Could you check a few things on this model? Use its own coordinates, in mm. Give positions to 0.01 mm unless a question says otherwise; leave off trailing zeros. Loops run counter-clockwise (first coordinate to the right, second up) from the corner with the lowest first, then second, coordinate; pieces in that order, holes last. Notation, with made-up numbers: (26, 41) - (43, 41) arc R23 ccw to (43, 69) - close; hole circle Ø1 at (52, 8.5). An arc over 180 degrees is marked (long way). One line per item, written item: value. Start each with the question number.
Q1. If I drill on line 1 (X direction, y = 59.7, z = 0.75); line 2 (Y direction, x = 0, z = 0.2); line 3 (X direction, y = 58.6, z = 0.2), over which ranges is the centre line in solid material (lowest first)? Write a range as from..to.
Q2. I'm going to push a flat-ended pin straight in: P1, Ø2, axis at x = 0, y = 59.56, coming from the +Z side. Where does the tip first touch, or does it pass through?
Q3. I want a section at A-A (x = 0). Please give me the cut outline in (y, z).
Q4. I want a section at B-B (z = 0.4). Please give me the cut outline in (x, y), then the cut area to 3 significant figures.
```python
from build123d import *

# Parameters (mm, degrees)
SKETCH1_W           = 119.309628318
SKETCH1_H           = 4.994236566
BOSS_EXTRUDE1_DEPTH = 1
SKETCH2_R           = 1.25
CUT_EXTRUDE1_DEPTH  = 1


with BuildPart() as part:
    # Sketch1 → Boss-Extrude1 (new body)
    with BuildSketch(Plane.XY):
        with Locations((0, 59.58360497)):
            Rectangle(SKETCH1_W, SKETCH1_H)
    extrude(amount=BOSS_EXTRUDE1_DEPTH)

    # Sketch2 → Cut-Extrude1 (cut)
    with BuildSketch(Plane.XY.offset(1)):
        with Locations((-54.300260115, 59.58360497)):
            Circle(SKETCH2_R)
        with Locations((0, 59.560111084)):
            Circle(SKETCH2_R)
        with Locations((54.300260115, 59.58360497)):
            Circle(SKETCH2_R)
    extrude(amount=-CUT_EXTRUDE1_DEPTH, mode=Mode.SUBTRACT)


solid = part.part
```
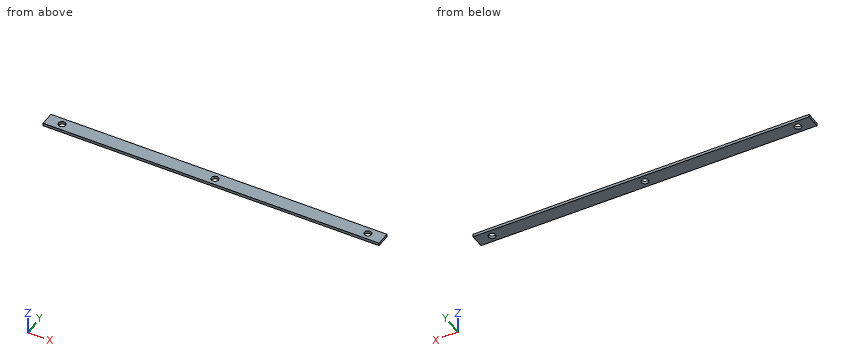
Worked answers:
1. line 1: x = -59.65..-55.54, -53.06..-1.24, 1.24..53.06, 55.54..59.65
1. line 2: y = 57.09..58.31, 60.81..62.08
1. line 3: x = -59.65..-55.07, -53.53..-0.8, 0.8..53.53, 55.07..59.65
2. P1: passes through
3. outline: (57.09, 0) - (58.31, 0) - (58.31, 1) - (57.09, 1) - close; (60.81, 0) - (62.08, 0) - (62.08, 1) - (60.81, 1) - close
4. outline: (-59.65, 57.09) - (59.65, 57.09) - (59.65, 62.08) - (-59.65, 62.08) - close; hole circle Ø2.5 at (-54.3, 59.58); hole circle Ø2.5 at (0, 59.56); hole circle Ø2.5 at (54.3, 59.58)
4. area: 581 mm²
